```python
from build123d import *

# Parameters (mm, degrees)
SKETCH1_R           = 5
BOSS_EXTRUDE1_DEPTH = 110
SKETCH2_W           = 10
SKETCH2_H           = 15
BOSS_EXTRUDE2_DEPTH = 20
SKETCH3_W           = 10
SKETCH3_H           = 15
BOSS_EXTRUDE3_DEPTH = 20
SKETCH4_R           = 5
CUT_EXTRUDE1_DEPTH  = 131.599578866


with BuildPart() as part:
    # Sketch1 → Boss-Extrude1 (new body)
    with BuildSketch(Plane.XY):
        Circle(SKETCH1_R)
    extrude(amount=BOSS_EXTRUDE1_DEPTH)

    # Sketch2 → Boss-Extrude2 (add)
    with BuildSketch(Plane(origin=(0, 0, 0), x_dir=(-1, 0, 0), z_dir=(0, 0, -1))):
        Rectangle(SKETCH2_W, SKETCH2_H)
    extrude(amount=BOSS_EXTRUDE2_DEPTH)

    # Sketch3 → Boss-Extrude3 (add)
    with BuildSketch(Plane.XY.offset(110)):
        Rectangle(SKETCH3_W, SKETCH3_H)
    extrude(amount=BOSS_EXTRUDE3_DEPTH)

    # Sketch4 → Cut-Extrude1 (cut, through all)
    with BuildSketch(Plane(origin=(5, 0, 0), x_dir=(0, 0, -1), z_dir=(1, 0, 0))):
        with Locations((12.5, 0)):
            Circle(SKETCH4_R)
        with Locations((-122.5, 0)):
            Circle(SKETCH4_R)
        with BuildLine():
            Line((12.5, -7.5), (27.957175819, -19.344646022))
            Line((27.957175819, -19.344646022), (25.412525065, 11.111642689))
            Line((25.412525065, 11.111642689), (12.5, 7.5))
            ThreePointArc((12.5, 7.5), (20, 0), (12.5, -7.5))
        make_face()
        with BuildLine():
            Line((-122.5, 7.5), (-386.499272389, 23.053021062))
            Line((-386.499272389, 23.053021062), (-390.004854727, -19.344646022))
            Line((-390.004854727, -19.344646022), (-122.5, -7.5))
            ThreePointArc((-122.5, -7.5), (-130, 0), (-122.5, 7.5))
        make_face()
    extrude(amount=-CUT_EXTRUDE1_DEPTH, mode=Mode.SUBTRACT)


solid = part.part
```
Build history of the part. All positions in model axes, mm. A direction names the side the tool comes from. Coordinates: 2 decimals unless noted, no trailing zeros. Order: outer loops, then holes, each group sorted by start corner. A loop starts at its lowest first (then second) coordinate and runs counter-clockwise, first axis right, second up. Notation, with made-up numbers: M 37,-9 L 77,-9 A15 cw 77,18 Z; hole C -33,-33.75 d10. An arc over 180 degrees is marked long. One line per question, with ' | ' between items. Start each with the question number.
1. Cut at A-A (x = 0). Write the cut outline in (y, z).
2. Wall check: line 1 along Z through (x, y) = (4.75, -0.25); line 2 along Z through (x, y) = (2.75, 4.25); line 3 along Y through (x, z) = (2.5, -12.5). Give the ranges that are in metal, low to high. Write a range as [from, to].
3. Cut at B-B (y = -2.5). Write the cut outline in (x, z), plus the area to 3 significant figures.
4. Cut at C-C (z = -9). Write the cut outline in (x, y), plus the area to 3 significant figures.
5. Cut at D-D (z = 81). Write the cut outline in (x, y), plus the area to 3 significant figures.
6. Mould opens along Y. For faces 1 (the face through (0, -7.5, 116)), 2 (the face through (0.07, 1.5, -17.27)), 3 (the face through (-1.08, -4.88, 54.23)) say: +Y half, -Y half, draft (parallel to the pull), parting line (faces both ways), or undercut.
7. Tool access for faces 4 (the face through (0.1, 5.5, 0)), 5 (the face through (-5, -1.8, 117.6)), 6 (the face through (0.1, -5.4, 0)): list every direction of +Z, -Z, +X, -X, +Y, -Y with a clear straight run to the whole face (end or side of a thin tool).
8. Flat gauge pins, fed straight in: P1, Ø1, axis at x = 2, z = 71.5, coming from the +Y side; P2, Ø2, axis at x = -0.5, z = 52.5, coming from the -Y side; P3, Ø6, axis at y = 5, z = 26, coming from the -X side. Where does each tip first touch, or does it go through?
The answers:
1) outline: M -7.5,-12.5 A7.5 ccw 7.5,-12.5 L 7.5,0 L 5,0 L 5,110 L 7.5,110 L 7.5,122.5 A7.5 ccw -7.5,122.5 L -7.5,110 L -5,110 L -5,0 L -7.5,0 Z; hole C 0,-12.5 d10; hole C 0,122.5 d10
2) line 1: z = [-20, -17.49], [-7.51, 117.51], [127.49, 130] | line 2: z = [-18.68, -15.13], [-9.87, 0], [110, 119.87], [125.13, 128.68] | line 3: y = [-7.5, -5], [5, 7.5]
3) outline: M -5,-19.57 L 5,-19.57 L 5,-16.83 L -5,-16.83 Z; M -5,-8.17 L 5,-8.17 L 5,0 L 4.33,0 L 4.33,110 L 5,110 L 5,118.17 L -5,118.17 L -5,110 L -4.33,110 L -4.33,0 L -5,0 Z; M -5,126.83 L 5,126.83 L 5,129.57 L -5,129.57 Z | area: 1,170 mm2
4) outline: M -5,-7.5 L 5,-7.5 L 5,-3.57 L -5,-3.57 Z; M -5,3.57 L 5,3.57 L 5,7.5 L -5,7.5 Z | area: 78.6 mm2
5) outline: C 0,0 d10 | area: 78.5 mm2
6) face 1: -Y half | face 2: undercut | face 3: parting line
7) face 4: +Y | face 5: +Z, -Z, -X, +Y, -Y | face 6: -Y
8) P1: stops at y = 4.77 | P2: stops at y = -5 | P3: stops at x = -4.58
